For this review, take the finished solid that the model builds, in its own axes (mm). A direction names the side the tool comes from. Give positions to 0.01 mm unless a question says otherwise; leave off trailing zeros. Write each loop counter-clockwise with the first axis right and the second up, starting at its lowest first coordinate (ties: lowest second). Pieces come first, ordered by that corner, then holes. Notation, with made-up numbers: M 70,47 L 82,47 A28 ccw 82,83 Z; hole C 73.25,3 d5. An arc over 180 degrees is marked long. Answer as a JSON object with one key per item and string values. Group by question number.
```python
from build123d import *

# Parameters (mm, degrees)
BOSS_EXTRUDE1_DEPTH = 15
SKETCH2_W           = 38.199379203
SKETCH2_H           = 20.357752988
CUT_EXTRUDE1_DEPTH  = 30
SKETCH3_W           = 25
SKETCH3_H           = 5
CUT_EXTRUDE2_DEPTH  = 30
BOSS_EXTRUDE3_START = 6
SKETCH4_R           = 2
BOSS_EXTRUDE3_DEPTH = 5
SKETCH5_R           = 3
CUT_EXTRUDE3_DEPTH  = 27
FILLET1_R           = 5
FILLET2_R           = 5


with BuildPart() as part:
    # Sketch1 → Boss-Extrude1 (new, symmetric)
    with BuildSketch(Plane.XY):
        Polygon((0, 0), (0, 5), (-15, 15), (-40, 15), (-40, 0), align=None)
    extrude(amount=BOSS_EXTRUDE1_DEPTH, both=True)

    # Sketch2 → Cut-Extrude1 (cut)
    with BuildSketch(Plane(origin=(0, 15, 0), x_dir=(1, 0, 0), z_dir=(0, 1, 0))):
        with Locations((-44.099689602, 22.178876494)):
            Rectangle(SKETCH2_W, SKETCH2_H)
        with Locations((-44.099689602, -22.178876494)):
            Rectangle(SKETCH2_W, SKETCH2_H)
    extrude(amount=-CUT_EXTRUDE1_DEPTH, mode=Mode.SUBTRACT)

    # Sketch3 → Cut-Extrude2 (cut)
    with BuildSketch(Plane(origin=(0, 15, 0), x_dir=(1, 0, 0), z_dir=(0, 1, 0))):
        with Locations((-27.5, -6.5)):
            Rectangle(SKETCH3_W, SKETCH3_H)
    extrude(amount=-CUT_EXTRUDE2_DEPTH, mode=Mode.SUBTRACT)

    # Sketch4 → Boss-Extrude3 (add)
    with BuildSketch(Plane.XY.offset(-15).offset(BOSS_EXTRUDE3_START)):
        with BuildLine():
            Line((-15, 15), (-32.226499019, 26.484332679))
            ThreePointArc((-32.226499019, 26.484332679), (-37.359289628, 26.732454201), (-40, 22.324081208))
            Line((-40, 22.324081208), (-40, 15))
            Line((-40, 15), (-15, 15))
        make_face()
        with Locations((-35, 22.324081208)):
            Circle(SKETCH4_R, mode=Mode.SUBTRACT)
    extrude(amount=BOSS_EXTRUDE3_DEPTH)

    # Sketch5 → Cut-Extrude3 (cut)
    with BuildSketch(Plane.XY.offset(12)):
        with Locations((-32.5, 7.5)):
            Circle(SKETCH5_R)
    extrude(amount=-CUT_EXTRUDE3_DEPTH, mode=Mode.SUBTRACT)

    # Fillet1
    fillet1_edges = [part.edges().sort_by_distance(p)[0] for p in [
        (-40, 0, 10.5),
        (-40, 15, 10.5),
    ]]
    fillet(fillet1_edges, radius=FILLET1_R)

    # Fillet2
    fillet2_edges = [part.edges().sort_by_distance(p)[0] for p in [
        (-40, 0, -4),
    ]]
    fillet(fillet2_edges, radius=FILLET2_R)


solid = part.part
```
Item 1: Consider section B-B (y = 21.5). Give the boundary of the cut face in (x, z).
Item 2: Consider section C-C (y = 7.5). Give the boundary of the cut face in (x, z).
Item 3: Insertion check: P1, Ø1.5, axis at y = 4, z = 6, coming from the -X side; P2, Ø10, axis at x = -28.5, y = 20.5, coming from the +Z side; P3, Ø8, axis at y = 18, z = 8.5, coming from the -X side. Each pin has a flat end and moves straight along its axis. Give the tip position at first contact, or say it passes through.
Item 4: Consider section D-D (x = -24.5). Give the boundary of the cut face in (y, z), plus the area to 3 significant figures.
Item 5: Machinability: for faces 1 (the flat face through (-25, 15, -11)), 2 (the flat face through (-15, 8, 7)), 3 (the cylindrical face through (-38, 14, 10)), which of the approach directions +Z, -Z, +X, -X, +Y, -Y give a long, thin tool a straight path to every point of the face, cutting with its end or side? Answer none if there is none.
Item 6: Consider section A-A (z = -5.5). Give the boundary of the cut face in (x, y), plus the area to 3 significant figures.
Item 7: To check wall thickness, follow probe 1 along Y at (x, z) = (-32.5, 9.75); probe 2 along Z at (x, y) = (-24, 13.25); probe 3 along Z at (x, y) = (-31.5, 12.25). State the ranges of each line that lie inside material, in increasing order.
Item 8: Draft analysis for pull direction Z (two halves, no side actions). For faces 4 (the flat face through (-18, 0, 0)), 5 (the flat face through (-15, 6, 15)), 6 (the flat face through (-28, 8, 4)), state which applies: released by +Z, released by -Z, zero draft, split by the parting line, or undercut.
Result set:
{
 "1": {"outline": "M -40,-9 L -36.82,-9 L -36.82,-4 L -40,-4 Z; M -33.18,-9 L -24.75,-9 L -24.75,-4 L -33.18,-4 Z"},
 "2": {"outline": "M -40,-12 L -35.5,-12 L -35.5,4 L -40,4 Z; M -40,9 L -35.5,9 L -35.5,12 L -40,12 Z; M -29.5,-12 L -25,-12 L -25,-15 L -3.75,-15 L -3.75,15 L -25,15 L -25,12 L -29.5,12 L -29.5,9 L -15,9 L -15,4 L -29.5,4 Z"},
 "3": {"P1": "stops at x = -15", "P2": "stops at z = -4", "P3": "stops at x = -37.96"},
 "4": {"outline": "M 0,-15 L 15,-15 L 15,-9 L 21.33,-9 L 21.33,-4 L 15,-4 L 15,4 L 0,4 Z; M 0,9 L 15,9 L 15,15 L 0,15 Z", "area": "407 mm^2"},
 "5": {"face 1": "-Z, +X, -X, +Y", "face 2": "-X, +Y, -Y", "face 3": "+Z, -X, +Y"},
 "6": {"outline": "M -40,5 A5 ccw -35,0 L 0,0 L 0,5 L -32.23,26.48 A5 ccw -40,22.32 Z; hole C -35,22.32 d4; hole C -32.5,7.5 d6", "area": "667 mm^2"},
 "7": {"probe 1": "y = 0 to 4.5, 10.5 to 15", "probe 2": "z = -15 to 4, 9 to 15", "probe 3": "z = -12 to 4, 9 to 12"},
 "8": {"face 4": "zero draft", "face 5": "released by +Z", "face 6": "undercut"}
}
